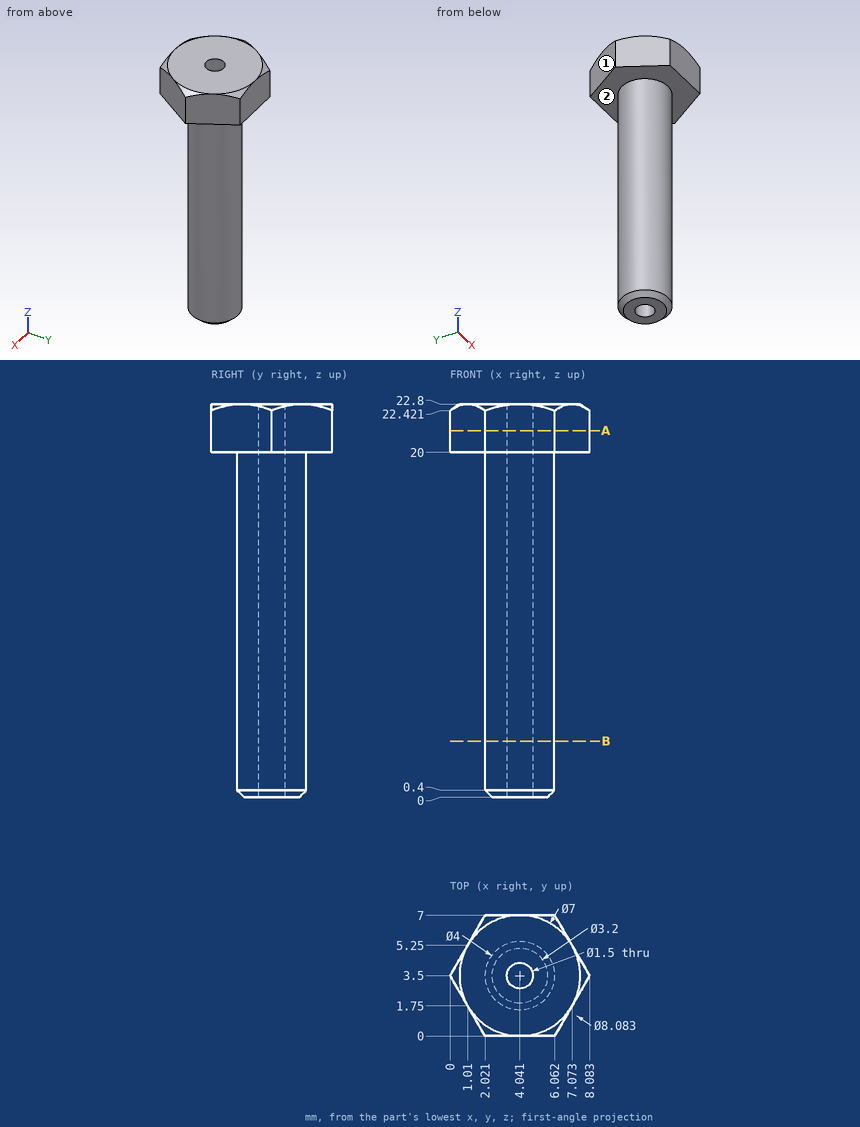
Geometry check sheet. Reference: drawing and pictorial views, mm from the part's lowest x, y, z. A direction names the side the tool comes from. Coordinates: 2 decimals unless noted, no trailing zeros. Write each loop counter-clockwise with the first axis right and the second up, starting at its lowest first coordinate (ties: lowest second). Pieces come first, ordered by that corner, then holes. Notation, with made-up numbers: (11.5, 15) - (27.5, 15) arc R8 ccw to (27.5, 27) - close; hole circle Ø2 at (80, 87.5). An arc over 180 degrees is marked (long way). One line per question, with ' | ' between items. Start each with the question number.
1. Material ranges on line 1 along X through (y, z) = (3.5, 17); line 2 along Y through (x, z) = (4, 4.5); line 3 along X through (y, z) = (4, 7.75) (1 decimal), recorded low to high.
2. Access from +Z, -Z, +X, -X, +Y, -Y to the whole of each face (thin tool, end or side, straight path). Record for the marked faces 1 and 2.
3. Gauge pin test, flat ends, axial feed: P1, Ø1, axis at x = 4.5, y = 1, coming from the -Z side; P2, Ø4, axis at y = 1, z = 19, coming from the -X side; P3, Ø1, axis at x = 2, z = 8, coming from the -Y side (1 decimal). Record the tip position at first contact, or that the pin passes through.
4. Section check A-A (z = 21.25). Enter the section's corners in (x, y).
5. Section check B-B (z = 3.25). Enter the section's corners in (x, y), plus the area to 3 significant figures.
Computed values:
1) line 1: 2.04 to 3.29, 4.79 to 6.04 | line 2: 1.5 to 2.75, 4.25 to 5.5 | line 3: 2.1 to 3.5, 4.6 to 6
2) face 1: +Z, -Z, -X, +Y | face 2: -Z
3) P1: z = 20 | P2: x = 0.44 | P3: y = 2.2
4) outline: (0, 3.5) - (2.02, 0) - (6.06, 0) - (8.08, 3.5) - (6.06, 7) - (2.02, 7) - close; hole circle Ø1.5 at (4.04, 3.5)
5) outline: circle Ø4 at (4.04, 3.5); hole circle Ø1.5 at (4.04, 3.5) | area: 10.8 mm²
